Build history of the part. All positions in model axes, mm. Give positions to 0.01 mm unless a question says otherwise; leave off trailing zeros. Order: outer loops, then holes, each group sorted by start corner. A loop starts at its lowest first (then second) coordinate and runs counter-clockwise, first axis right, second up. Notation, with made-up numbers: (32, -3.5) - (39, -3.5) arc R22 cw to (39, 20.5) - close; hole circle Ø9 at (48, 84). An arc over 180 degrees is marked (long way). Answer in a Markdown table with one row per item.
```python
from build123d import *

# Parameters (mm, degrees)
SKETCH_1_W          = 10
SKETCH_1_H          = 6
EXTRUDE_1_DEPTH     = 10
SKETCH_2_R          = 1.5
CUT_EXTRUDE_1_DEPTH = 16.362291496
SKETCH_4_R          = 1.5
CUT_EXTRUDE_2_DEPTH = 16.362291496
SKETCH_3_R          = 1.5
CUT_EXTRUDE_3_DEPTH = 16.362291496


with BuildPart() as part:
    # 草图1 → 凸台-拉伸1 (new body)
    with BuildSketch(Plane(origin=(0, 0, 0), x_dir=(1, 0, 0), z_dir=(0, 1, 0))):
        with Locations((5, 3)):
            Rectangle(SKETCH_1_W, SKETCH_1_H)
    extrude(amount=EXTRUDE_1_DEPTH)

    # 草图2 → 切除-拉伸1 (cut, through all)
    with BuildSketch(Plane.XY):
        with Locations((5, 5)):
            Circle(SKETCH_2_R)
    extrude(amount=-CUT_EXTRUDE_1_DEPTH, mode=Mode.SUBTRACT)

    # 草图4 → 切除-拉伸2 (cut, through all)
    with BuildSketch(Plane(origin=(0, 10, 0), x_dir=(1, 0, 0), z_dir=(0, 1, 0))):
        with Locations(Location((5, 3, 0), (0, 0, 270))):
            Circle(SKETCH_4_R)
    extrude(amount=-CUT_EXTRUDE_2_DEPTH, mode=Mode.SUBTRACT)

    # 草图3 → 切除-拉伸3 (cut, through all)
    with BuildSketch(Plane(origin=(10, 0, 0), x_dir=(0, 0, -1), z_dir=(1, 0, 0))):
        with Locations((3, 5)):
            Circle(SKETCH_3_R)
    extrude(amount=-CUT_EXTRUDE_3_DEPTH, mode=Mode.SUBTRACT)


solid = part.part
```
1. Probe line 1 (Z direction, x = 8.9, y = 5); line 2 (Y direction, x = 8.1, z = -3). List the from-to ranges inside material, lowest first.
Check result:
| item | result |
|---|---|
| line 1 | z = -6 to -4.5, -1.5 to 0 |
| line 2 | y = 0 to 3.5, 6.5 to 10 |
2. Cut at A-A on y = 5. Write the cut outline in (x, z).
Check result:
| item | result |
|---|---|
| outline | (0, -6) - (3.5, -6) - (3.5, -4.5) - (0, -4.5) - close; (0, -1.5) - (3.5, -1.5) - (3.5, 0) - (0, 0) - close; (6.5, -6) - (10, -6) - (10, -4.5) - (6.5, -4.5) - close; (6.5, -1.5) - (10, -1.5) - (10, 0) - (6.5, 0) - close |
3. Cut at D-D on z = -0.6. Write the cut outline in (x, y).
Check result:
| item | result |
|---|---|
| outline | (0, 0) - (10, 0) - (10, 10) - (0, 10) - close; hole circle Ø3 at (5, 5) |
4. Cut at C-C on x = 6.75. Write the cut outline in (y, z).
Check result:
| item | result |
|---|---|
| outline | (0, -6) - (10, -6) - (10, 0) - (0, 0) - close; hole circle Ø3 at (5, -3) |
5. Cut at B-B on z = -3. Write the cut outline in (x, y).
Check result:
| item | result |
|---|---|
| outline | (0, 0) - (3.5, 0) - (3.5, 3.5) - (0, 3.5) - close; (0, 6.5) - (3.5, 6.5) - (3.5, 10) - (0, 10) - close; (6.5, 0) - (10, 0) - (10, 3.5) - (6.5, 3.5) - close; (6.5, 6.5) - (10, 6.5) - (10, 10) - (6.5, 10) - close |
6. Two-plate mould, pull along Z, no slides. Class faces 1 (the face through (2, 5.07, -1.5)), 2 (the face through (3.8, 3.8, 0)), 3 (the face through (0, 3.8, -1.6)), 4 (the face through (3.8, 3.8, -6)): +Z half, -Z half, draft (parallel to the pull), parting line (faces both ways), or undercut.
Check result:
| item | result |
|---|---|
| face 1 | undercut |
| face 2 | +Z half |
| face 3 | draft |
| face 4 | -Z half |
